Study the drawing (mm; zero at the part's minimum x, y, z) and answer. Coordinates: 2 decimals unless noted, no trailing zeros. Order: outer loops, then holes, each group sorted by start corner. A loop starts at its lowest first (then second) coordinate and runs counter-clockwise, first axis right, second up. Notation, with made-up numbers: M -8.5,-19 L 42.5,-19 A17 cw 42.5,8 Z; hole C 22.5,77.25 d9. An arc over 180 degrees is marked long. Put each result on its own line as item: value.
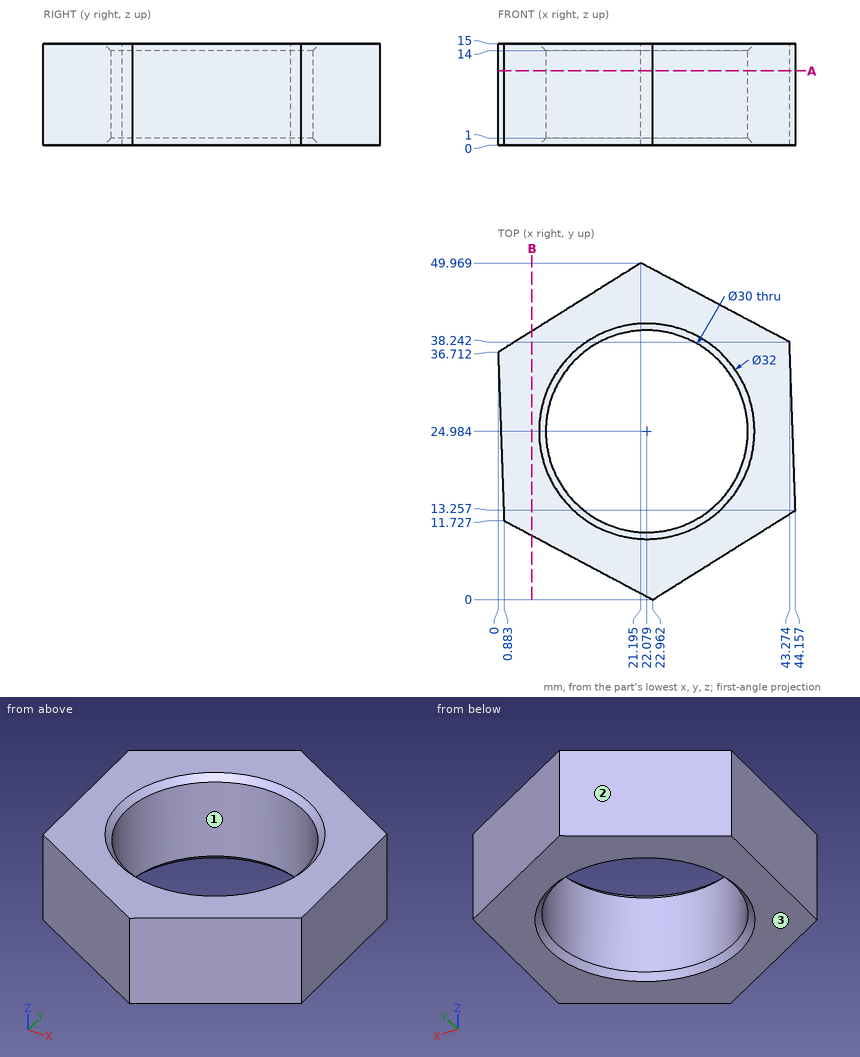
Q1. Find section A-A on z = 11. Write down the section's boundary in (x, y) (1 decimal), plus the area to 3 significant figures.
Answers below:
outline: M 0,36.7 L 0.9,11.7 L 23,0 L 44.2,13.3 L 43.3,38.2 L 21.2,50 Z; hole C 22.1,25 d30
area: 917 mm^2
Q2. Find section B-B on x = 5. Write down the section's boundary in (y, z).
Answers below:
outline: M 9.54,0 L 39.84,0 L 39.84,15 L 9.54,15 Z
Q3. Consider line 1 along Y through (x, z) = (9, 7.5) (1 decimal); line 2 along Y through (x, z) = (16.5, 6.25); line 3 along X through (y, z) = (36, 9) (1 decimal). Determine where each line is inside the solid, lowest interval first.
Answers below:
line 1: y = 7.4 to 17.6, 32.3 to 42.3
line 2: y = 3.43 to 11.06, 38.91 to 47.03
line 3: x = 0 to 11.9, 32.3 to 43.4
Q4. For a pull along Y with two mould halves and no side action, classify the marked faces 1, 2 and 3 as +Y half, -Y half, draft (parallel to the pull), parting line (faces both ways), or undercut.
Answers below:
face 1: undercut
face 2: +Y half
face 3: draft
Q5. Given pin 1 (8 mm diameter, centred on y = 28.5, z = 12.5, fed in from +X); pin 2 (24 mm diameter, centred on x = 22.08, y = 24.98, fed in from -Z); pin 3 (6 mm diameter, centred on x = 16.5, y = 41.5, fed in from -Z); pin 4 (5 mm diameter, centred on x = 37, z = 8, fed in from -Y), each flat-ended and moving along its own axis, determine where each tip first touches the part or whether it passes through.
Answers below:
pin 1: stops at x = 43.76
pin 2: passes through
pin 3: stops at z = 0
pin 4: stops at y = 7.22
